Build history of the part. All positions in model axes, mm. Face numbers are marked on the shaded views. A direction names the side the tool comes from. Coordinates: 2 decimals unless noted, no trailing zeros. Loops run counter-clockwise (first coordinate to the right, second up) from the corner with the lowest first, then second, coordinate; pieces in that order, holes last. Notation, with made-up numbers: (54.25, -20) - (85.25, -20) arc R27 cw to (85.25, 12) - close; hole circle Ø5 at (76, -1.75). An arc over 180 degrees is marked (long way). One line per item, written item: value.
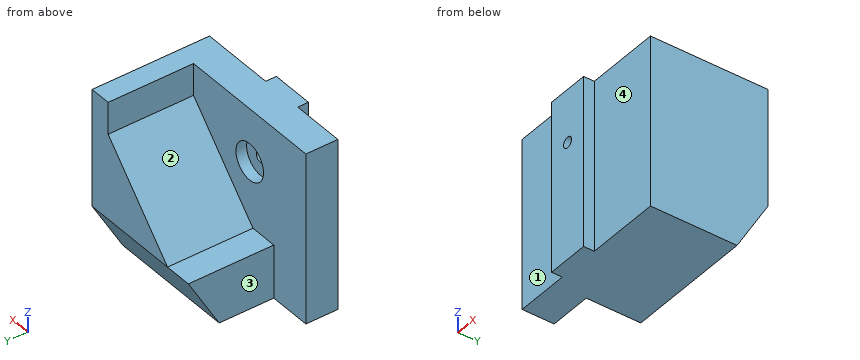
```python
from build123d import *

# Parameters (mm, degrees)
BASE_PROFILE_SKETCH_W       = 80
BASE_PROFILE_SKETCH_H       = 20
BASE_BLOCK_DEPTH            = 80
UNDERSIDE_SLOT_SKETCH_W     = 25
UNDERSIDE_SLOT_SKETCH_H     = 5
UNDERSIDE_SLOT_SKETCH_W_2   = 35
UNDERSIDE_SLOT_DEPTH        = 80
UPRIGHT_WALL_SKETCH_W       = 10
UPRIGHT_WALL_SKETCH_H       = 80
UPRIGHT_WALL_DEPTH          = 40
SIDE_BLOCK_DEPTH            = 40
WALL_CHAMFER_25X30DEG_SIZE  = 25
WALL_CHAMFER_25X30DEG_SIZE2 = 14.43375673
COUNTERBORE_SKETCH_R        = 8.583879332
COUNTERBORE_RECESS_DEPTH    = 5
HOLE_SKETCH_R               = 2.5
HOLE_DIA5_DEPTH             = 22


with BuildPart() as part:
    # Base Profile Sketch → Base Block (new body)
    with BuildSketch(Plane.XY):
        Rectangle(BASE_PROFILE_SKETCH_W, BASE_PROFILE_SKETCH_H)
    extrude(amount=BASE_BLOCK_DEPTH)

    # Underside Slot Sketch → Underside Slot (cut)
    with BuildSketch(Plane.XY.offset(80)):
        with Locations((-27.5, -7.5)):
            Rectangle(UNDERSIDE_SLOT_SKETCH_W, UNDERSIDE_SLOT_SKETCH_H)
        with Locations((22.5, -7.5)):
            Rectangle(UNDERSIDE_SLOT_SKETCH_W_2, UNDERSIDE_SLOT_SKETCH_H)
    extrude(amount=-UNDERSIDE_SLOT_DEPTH, mode=Mode.SUBTRACT)

    # Upright Wall Sketch → Upright Wall (add)
    with BuildSketch(Plane(origin=(0, 10, 0), x_dir=(1, 0, 0), z_dir=(0, 1, 0))):
        with Locations((35, -40)):
            Rectangle(UPRIGHT_WALL_SKETCH_W, UPRIGHT_WALL_SKETCH_H)
    extrude(amount=UPRIGHT_WALL_DEPTH)

    # Side Block Sketch → Side Block (add)
    with BuildSketch(Plane(origin=(0, 10, 0), x_dir=(1, 0, 0), z_dir=(0, 1, 0))):
        Polygon((-20, 0), (-20, -25), (-7.006583052, -25), (30, -65), (30, 0), align=None)
    extrude(amount=SIDE_BLOCK_DEPTH)

    # Wall Chamfer 25x30deg
    wall_chamfer_25x30deg_edges = [part.edges().sort_by_distance(p)[0] for p in [
        (10, 50, 0),
    ]]
    wall_chamfer_25x30deg_side = [part.faces().sort_by_distance(p)[0] for p in [
        (16.961219392, 50, 27.237680119),
    ]]
    chamfer(wall_chamfer_25x30deg_edges, length=WALL_CHAMFER_25X30DEG_SIZE, length2=WALL_CHAMFER_25X30DEG_SIZE2, reference=wall_chamfer_25x30deg_side[0])

    # Counterbore Sketch → Counterbore Recess (cut)
    with BuildSketch(Plane(origin=(0, 10, 0), x_dir=(1, 0, 0), z_dir=(0, 1, 0))):
        with Locations(Location((-5, -55, 0), (0, 0, 270))):
            Circle(COUNTERBORE_SKETCH_R)
    extrude(amount=-COUNTERBORE_RECESS_DEPTH, mode=Mode.SUBTRACT)

    # Hole Sketch → Hole Dia5 (cut)
    with BuildSketch(Plane(origin=(0, 5, 0), x_dir=(1, 0, 0), z_dir=(0, 1, 0))):
        with Locations(Location((-5, -55, 0), (0, 0, 270))):
            Circle(HOLE_SKETCH_R)
    extrude(amount=-HOLE_DIA5_DEPTH, mode=Mode.SUBTRACT)


solid = part.part
```
Item 1: Probe probe 1 along X at (y, z) = (7.3, 55); probe 2 along X at (y, z) = (-6.5, 55); probe 3 along Y at (x, z) = (2, 68.5). List the from-to ranges inside material, lowest first. Write a range as from..to.
Check result:
probe 1: x = -40..-13.58, 3.58..40
probe 2: x = -15..-7.5, -2.5..5
probe 3: y = -10..10
Item 2: Cut at D-D, the plane x = 31.5. Write the cut outline in (y, z), then the cut area to 3 significant figures.
Check result:
outline: (-5, 0) - (35.57, 0) - (50, 25) - (50, 80) - (-5, 80) - close
area: 4,220 mm^2
Item 3: Cut at C-C, the plane z = 55. Write the cut outline in (x, y), then the cut area to 3 significant figures.
Check result:
outline: (-40, -5) - (-15, -5) - (-15, -10) - (-7.5, -10) - (-7.5, 5) - (-13.58, 5) - (-13.58, 10) - (-40, 10) - close; (-2.5, -10) - (5, -10) - (5, -5) - (40, -5) - (40, 50) - (20.75, 50) - (20.75, 10) - (3.58, 10) - (3.58, 5) - (-2.5, 5) - close
area: 1,910 mm^2
Item 4: Drop flat-ended pins along their axis: P1, Ø8, axis at x = 15.5, z = 68.5, coming from the +Y side; P2, Ø1.5, axis at y = -8.5, z = 28.5, coming from the +X side; P3, Ø1.5, axis at y = -8, z = 57, coming from the -X side. Give the stop position or say it passes through.
Check result:
P1: stops at y = 10
P2: stops at x = 5
P3: stops at x = -15
Item 5: Tool access for the marked faces 1, 2, 3 and 4: list every direction of +Z, -Z, +X, -X, +Y, -Y with a clear straight run to the whole face (end or side of a thin tool).
Check result:
face 1: +Z, -Z, -X, -Y
face 2: +Z, -X, +Y
face 3: +Z, -Z, -X, +Y
face 4: +Z, -Z, +X, -Y
Item 6: Cut at B-B, the plane y = 26.5. Write the cut outline in (x, z), then the cut area to 3 significant figures.
Check result:
outline: (-20, 0) - (40, 0) - (40, 80) - (30, 80) - (30, 65) - (-7.01, 25) - (-20, 25) - close
area: 2,790 mm^2
Item 7: Cut at A-A, the plane z = 69.5. Write the cut outline in (x, y), then the cut area to 3 significant figures.
Check result:
outline: (-40, -5) - (-15, -5) - (-15, -10) - (5, -10) - (5, -5) - (40, -5) - (40, 50) - (30, 50) - (30, 10) - (-40, 10) - close
area: 1,700 mm^2
